For this review, take the finished solid that the model builds, in its own axes (mm). A direction names the side the tool comes from. Coordinates: 2 decimals unless noted, no trailing zeros. Order: outer loops, then holes, each group sorted by start corner. A loop starts at its lowest first (then second) coordinate and runs counter-clockwise, first axis right, second up. Notation, with made-up numbers: (13.25, 19) -> (72.25, 19) arc R9 cw to (72.25, 32) -> close; hole circle Ø10 at (52, 61.25). An arc over 180 degrees is marked (long way). Answer as a JSON object with one key per item and string values. Group by question number.
1) Add section D-D, the plane y = -50. Write out the cut boundary in (x, z), then the cut area to 3 significant figures.
2) Add section B-B, the plane z = 32. Write out the cut boundary in (x, y).
3) Add section A-A, the plane y = -6.5. Write out the cut boundary in (x, z), then the cut area to 3 significant figures.
4) Wall thickness on L1, parallel to Z at x = 0, y = -7.5; L2, parallel to Z at x = 2, y = 47.5; L3, parallel to Z at x = 27, y = 44.5: over which ranges is each line inside the solid? List them lowest first.
5) Draft analysis for pull direction X (two halves, no side actions). For faces 4 (the cylindrical face through (-16.484, 0.725, 59.72)), 5 (the flat face through (23, 1, 92.5)), 6 (the conical face through (-0.25, -2.46, 50.23)), state which applies: +X half, -X half, draft (parallel to the pull), parting line (faces both ways), or undercut.
6) Machinability: for faces 1 (the cylindrical face through (2.17, -9.76, -44.86)), 2 (the cylindrical face through (0.8, -8.57, 52.44)), 3 (the flat face through (2, 13.5, 52)), which of the approach directions +Z, -Z, +X, -X, +Y, -Y give a long, thin tool a straight path to every point of the face, cutting with its end or side? Answer none if there is none.
7) For pin 1 (1.5 mm diameter, centred on x = -16, y = -14.5, fed in from -Z); pin 2 (11 mm diameter, centred on x = 24.5, y = -30, fed in from +Z); pin 3 (4 mm diameter, centred on x = 0, z = 50.5, fed in from -Y); pin 4 (1.6 mm diameter, centred on y = -18, z = 93, fed in from +X), all flat-tipped, find the tip position at first contact; note any pin that passes through.
8) Add section C-C, the plane x = -6. Write out the cut boundary in (y, z).
from build123d import *

# Parameters (mm, degrees)
SKETCH_1_R          = 15
EXTRUDE_1_DEPTH     = 40
SKETCH_2_R          = 16.5
EXTRUDE_2_DEPTH     = 40
SKETCH_3_R          = 12.5
EXTRUDE_3_DEPTH     = 35
SKETCH_4_R          = 10
EXTRUDE_4_DEPTH     = 20
SKETCH_5_W          = 60
SKETCH_5_H          = 140
EXTRUDE_5_DEPTH     = 14
SKETCH_6_W          = 14
SKETCH_6_H          = 140
CUT_EXTRUDE_1_DEPTH = 1.5
SKETCH_7_W          = 13
SKETCH_7_H          = 3
CUT_EXTRUDE_2_DEPTH = 10


with BuildPart() as part:
    # 草图1 → 凸台-拉伸1 (new body)
    with BuildSketch(Plane.XY):
        Circle(SKETCH_1_R)
    extrude(amount=EXTRUDE_1_DEPTH)

    # 草图2 → 凸台-拉伸2 (add)
    with BuildSketch(Plane.XY.offset(40)):
        Circle(SKETCH_2_R)
    extrude(amount=EXTRUDE_2_DEPTH)

    # 草图3 → 凸台-拉伸3 (add)
    with BuildSketch(Plane(origin=(0, 0, 0), x_dir=(-1, 0, 0), z_dir=(0, 0, -1))):
        Circle(SKETCH_3_R)
    extrude(amount=EXTRUDE_3_DEPTH)

    # 草图4 → 凸台-拉伸4 (add)
    with BuildSketch(Plane(origin=(0, 0, -35), x_dir=(-1, 0, 0), z_dir=(0, 0, -1))):
        Circle(SKETCH_4_R)
    extrude(amount=EXTRUDE_4_DEPTH)

    # 草图5 → 凸台-拉伸5 (add)
    with BuildSketch(Plane.XY.offset(80)):
        Rectangle(SKETCH_5_W, SKETCH_5_H)
    extrude(amount=EXTRUDE_5_DEPTH)

    # 草图6 → 切除-拉伸1 (cut)
    with BuildSketch(Plane.XY.offset(94)):
        with Locations((23, 0)):
            Rectangle(SKETCH_6_W, SKETCH_6_H)
    extrude(amount=-CUT_EXTRUDE_1_DEPTH, mode=Mode.SUBTRACT)

    # 草图7 → 切除-拉伸2 (cut, symmetric)
    with BuildSketch(Plane(origin=(0, 0, 0), x_dir=(0, 0, -1), z_dir=(1, 0, 0))):
        with Locations((-50.5, 15)):
            Rectangle(SKETCH_7_W, SKETCH_7_H)
    cut_extrude_2 = extrude(amount=CUT_EXTRUDE_2_DEPTH, both=True, mode=Mode.SUBTRACT)

    # 镜向1: 切除-拉伸2 across plane
    add(cut_extrude_2.mirror(Plane.ZX), mode=Mode.SUBTRACT)

    # 草图8 → M5 螺纹孔1 (revolve, cut)
    with BuildSketch(Plane(origin=(0, 13.5, 50.5), x_dir=(0, 0, 1), z_dir=(1, 0, 0))):
        Polygon((0, 0), (0, 11.2618073), (2.1, 10), (2.1, 0), align=None)
    hole_wizard_m5_1 = revolve(axis=Axis((0, 19.85, 50.5), (0, -1, 0)), mode=Mode.SUBTRACT)

    # 镜向2: M5 螺纹孔1 across plane
    add(hole_wizard_m5_1.mirror(Plane.ZX), mode=Mode.SUBTRACT)


solid = part.part
Output values:
{
 "1": {"outline": "(-30, 80) -> (30, 80) -> (30, 92.5) -> (16, 92.5) -> (16, 94) -> (-30, 94) -> close", "area": "819 mm²"},
 "2": {"outline": "circle Ø30 at (0, 0)"},
 "3": {"outline": "(-30, 80) -> (-15.17, 80) -> (-15.17, 40) -> (-13.52, 40) -> (-13.52, 0) -> (-10.68, 0) -> (-10.68, -35) -> (-7.6, -35) -> (-7.6, -55) -> (7.6, -55) -> (7.6, -35) -> (10.68, -35) -> (10.68, 0) -> (13.52, 0) -> (13.52, 40) -> (15.17, 40) -> (15.17, 80) -> (30, 80) -> (30, 92.5) -> (16, 92.5) -> (16, 94) -> (-30, 94) -> close; hole circle Ø4.2 at (0, 50.5)", "area": "4,150 mm²"},
 "4": {"L1": "z = -55 to 48.4, 52.6 to 94", "L2": "z = 80 to 94", "L3": "z = 80 to 92.5"},
 "5": {"face 4": "parting line", "face 5": "draft", "face 6": "undercut"},
 "6": {"face 1": "-Z", "face 2": "-Y", "face 3": "+X, -X, +Y"},
 "7": {"pin 1": "stops at z = 80", "pin 2": "stops at z = 92.5", "pin 3": "stops at y = -3.44", "pin 4": "stops at x = 30"},
 "8": {"outline": "(-70, 80) -> (-15.37, 80) -> (-15.37, 57) -> (-13.5, 57) -> (-13.5, 44) -> (-15.37, 44) -> (-15.37, 40) -> (-13.75, 40) -> (-13.75, 0) -> (-10.97, 0) -> (-10.97, -35) -> (-8, -35) -> (-8, -55) -> (8, -55) -> (8, -35) -> (10.97, -35) -> (10.97, 0) -> (13.75, 0) -> (13.75, 40) -> (15.37, 40) -> (15.37, 44) -> (13.5, 44) -> (13.5, 57) -> (15.37, 57) -> (15.37, 80) -> (70, 80) -> (70, 94) -> (-70, 94) -> close"}
}
